Could you check a few things on this drawing? It's one solid part, dimensions in mm from its lowest x, y, z. Give positions to 0.01 mm unless a question says otherwise; leave off trailing zeros. Write each loop counter-clockwise with the first axis right and the second up, starting at its lowest first coordinate (ties: lowest second). Pieces come first, ordered by that corner, then holes.
1. Suppose I cut it at C-C (z = 11). Please give me the cut outline in (x, y).
2. Suppose I cut it at B-B (x = 140). Please give me the cut outline in (y, z).
3. If I drill on probe 1 along Y at (x, z) = (140, 13.25); probe 2 along Y at (x, z) = (88, 19.5); probe 3 along X at (y, z) = (106.5, 14.75), over which ranges is the centre line in solid material (lowest first)?
4. Suppose I cut it at A-A (y = 60). Please give me the cut outline in (x, z).
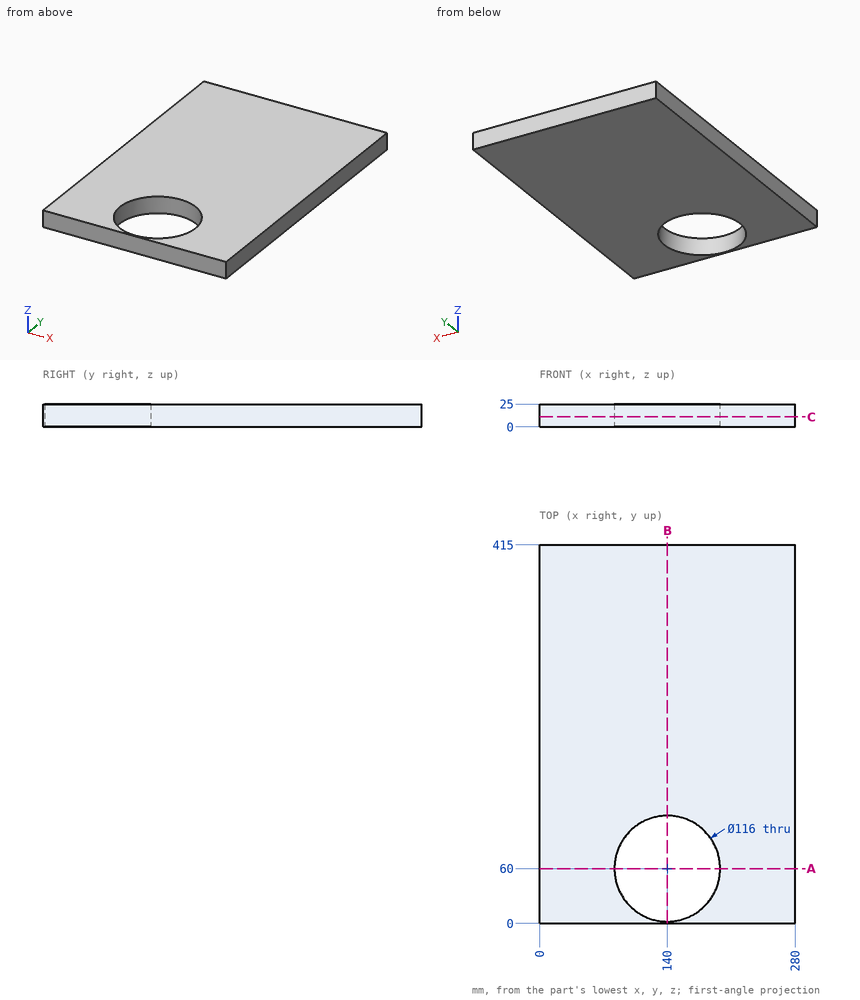
Checks:
1. outline: (0, 0) - (280, 0) - (280, 415) - (0, 415) - close; hole circle Ø116 at (140, 60)
2. outline: (0, 0) - (2, 0) - (2, 25) - (0, 25) - close; (118, 0) - (415, 0) - (415, 25) - (118, 25) - close
3. probe 1: y = 0 to 2, 118 to 415
3. probe 2: y = 0 to 34.31, 85.69 to 415
3. probe 3: x = 0 to 105.33, 174.67 to 280
4. outline: (0, 0) - (82, 0) - (82, 25) - (0, 25) - close; (198, 0) - (280, 0) - (280, 25) - (198, 25) - close
